Study the drawing (mm; zero at the part's minimum x, y, z) and answer. A direction names the side the tool comes from. Coordinates: 2 decimals unless noted, no trailing zeros. Write each loop counter-clockwise with the first axis right and the second up, starting at its lowest first coordinate (ties: lowest second). Pieces come first, ordered by that corner, then holes. Notation, with made-up numbers: M -26.5,82.25 L 5.5,82.25 A15 cw 5.5,103.25 Z; hole C -26,-40 d4. An arc over 180 degrees is marked long. Answer as CSV lines item,"result". Start each with the question number.
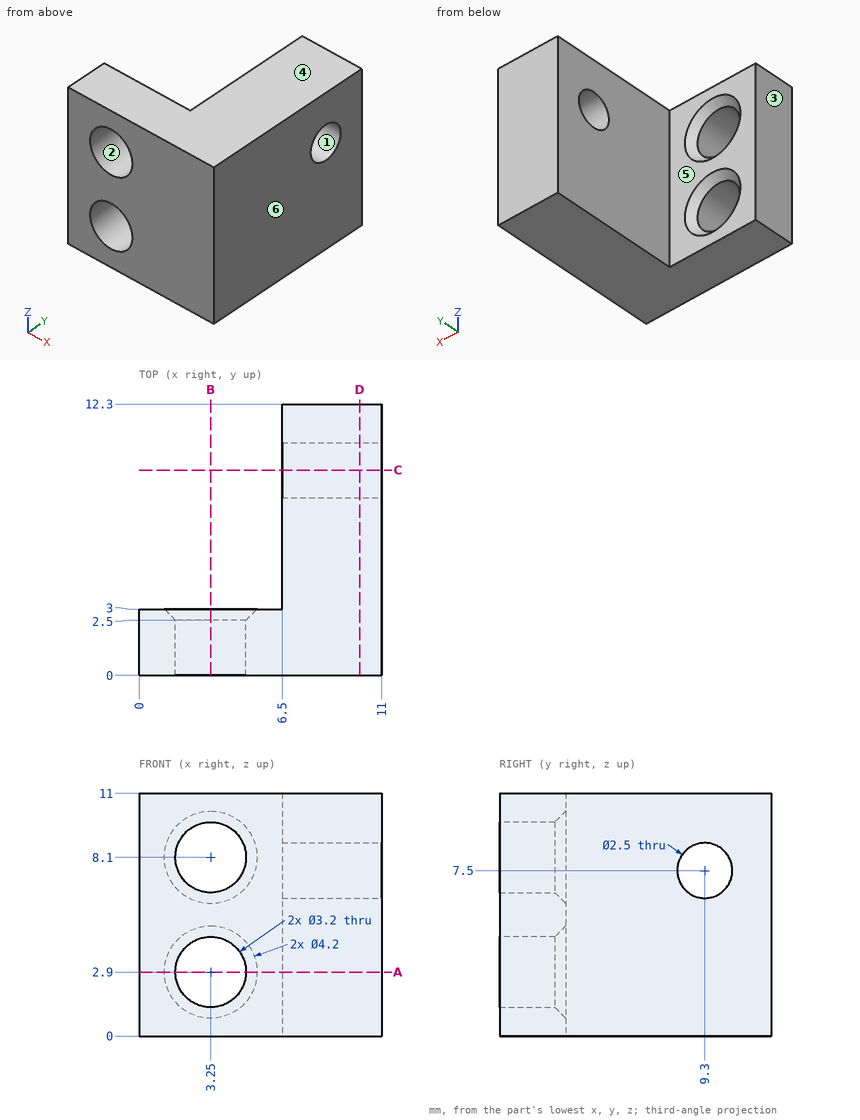
1) The part is cut by section A-A (z = 2.9). Determine the outline of the cut face in (x, y), then the cut area to 3 significant figures.
2) The part is cut by section C-C (y = 9.3). Determine the outline of the cut face in (x, z).
3) The part is cut by section B-B (x = 3.25). Determine the outline of the cut face in (y, z).
4) For a pull along Z with two mould halves and no side action, classify the marked faces 1, 2, 3 and 4 as +Z half, -Z half, draft (parallel to the pull), parting line (faces both ways), or undercut.
5) Each of these flat-tipped pins is pushed along its axis until it touches: P1, Ø5, axis at y = 10, z = 7, coming from the -X side; P2, Ø2, axis at x = 3.5, z = 5, coming from the +Y side; P3, Ø3, axis at x = 3.5, z = 2.5, coming from the +Y side. Where does it stop, or does it pass through?
6) The part is cut by section D-D (x = 10). Determine the outline of the cut face in (y, z).
7) Which of the six approach directions +Z, -Z, +X, -X, +Y, -Y give full straight-line access (tool end or side, diameter ignored) to the marked faces 5 and 6?
8) Find the intervals of material crossed by line 1 (X direction, y = 1.9, z = 8.1); line 2 (X direction, y = 10, z = 4.5); line 3 (Y direction, x = 2.25, z = 5.5), in increasing order. Write a range as from..to.
Completed:
1,outline,"M 0,0 L 1.65,0 L 1.65,2.5 L 1.15,3 L 0,3 Z; M 4.85,0 L 11,0 L 11,12.3 L 6.5,12.3 L 6.5,3 L 5.35,3 L 4.85,2.5 Z"
1,area,"65.0 mm²"
2,outline,"M 6.5,0 L 11,0 L 11,6.25 L 6.5,6.25 Z; M 6.5,8.75 L 11,8.75 L 11,11 L 6.5,11 Z"
3,outline,"M 0,0 L 3,0 L 3,0.8 L 2.5,1.3 L 0,1.3 Z; M 0,4.5 L 2.5,4.5 L 3,5 L 3,6 L 2.5,6.5 L 0,6.5 Z; M 0,9.7 L 2.5,9.7 L 3,10.2 L 3,11 L 0,11 Z"
4,face 1,"undercut"
4,face 2,"undercut"
4,face 3,"draft"
4,face 4,"+Z half"
5,P1,"x = 6.5"
5,P2,"y = 3"
5,P3,"y = 2.87"
6,outline,"M 0,0 L 12.3,0 L 12.3,11 L 0,11 Z; hole C 9.3,7.5 d2.5"
7,face 5,"+Z, -Z, -X, +Y"
7,face 6,"+Z, -Z, +X, +Y, -Y"
8,line 1,"0..1.65, 4.85..11"
8,line 2,"6.5..11"
8,line 3,"0..3"
